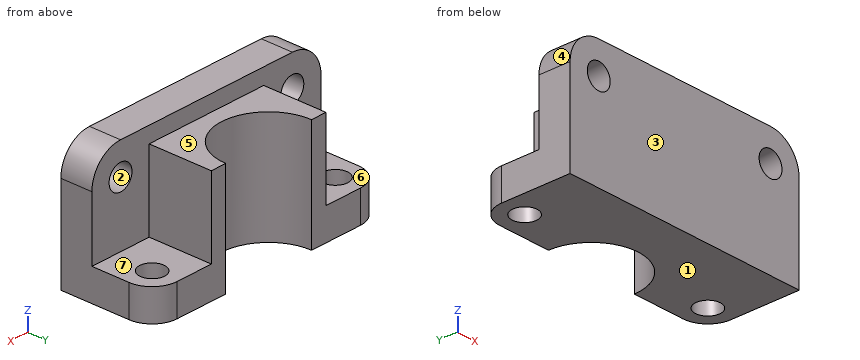
from build123d import *

# Parameters (mm, degrees)
BASE_PLATE_SKETCH_W       = 80
BASE_PLATE_SKETCH_H       = 40
BASE_PLATE_80X40X10_DEPTH = 10
BASE_CORNER_FILLETS_R10_R = 10
SADDLE_BLOCK_DEPTH        = 35
LUG_PROFILE_SKETCH_W      = 20
LUG_PROFILE_SKETCH_H      = 20
UPRIGHT_LUGS_DEPTH        = 10
LUG_TOP_FILLETS_R8_R      = 8
LUG_HOLE_SKETCH_R         = 4
LUG_HOLES_8_DEPTH         = 62
BASE_HOLE_SKETCH_R        = 4
BASE_HOLES_8_DEPTH        = 62


with BuildPart() as part:
    # Base Plate Sketch → Base Plate 80x40x10 (new body)
    with BuildSketch(Plane(origin=(0, 0, 0), x_dir=(1, 0, 0), z_dir=(0, 1, 0))):
        Rectangle(BASE_PLATE_SKETCH_W, BASE_PLATE_SKETCH_H)
    extrude(amount=BASE_PLATE_80X40X10_DEPTH)

    # Base Corner Fillets R10
    base_corner_fillets_r10_edges = [part.edges().sort_by_distance(p)[0] for p in [
        (40, 5, 20),
        (-40, 5, 20),
    ]]
    fillet(base_corner_fillets_r10_edges, radius=BASE_CORNER_FILLETS_R10_R)

    # Saddle Block Sketch → Saddle Block (add)
    with BuildSketch(Plane(origin=(0, 0, -20), x_dir=(-1, 0, 0), z_dir=(0, 0, -1))):
        with BuildLine():
            Line((-20, 10), (20, 10))
            Line((20, 10), (20, 30))
            Line((20, 30), (15, 30))
            ThreePointArc((15, 30), (0, 15), (-15, 30))
            Line((-15, 30), (-20, 30))
            Line((-20, 30), (-20, 10))
        make_face()
    extrude(amount=-SADDLE_BLOCK_DEPTH)

    # Lug Profile Sketch → Upright Lugs (add)
    with BuildSketch(Plane(origin=(0, 0, -20), x_dir=(-1, 0, 0), z_dir=(0, 0, -1))):
        with Locations((-30, 20)):
            Rectangle(LUG_PROFILE_SKETCH_W, LUG_PROFILE_SKETCH_H)
        with Locations((30, 20)):
            Rectangle(LUG_PROFILE_SKETCH_W, LUG_PROFILE_SKETCH_H)
    extrude(amount=-UPRIGHT_LUGS_DEPTH)

    # Lug Top Fillets R8
    lug_top_fillets_r8_edges = [part.edges().sort_by_distance(p)[0] for p in [
        (40, 30, -15),
        (-40, 30, -15),
    ]]
    fillet(lug_top_fillets_r8_edges, radius=LUG_TOP_FILLETS_R8_R)

    # Lug Hole Sketch → Lug Holes Ø8 (cut)
    with BuildSketch(Plane(origin=(0, 0, -20), x_dir=(-1, 0, 0), z_dir=(0, 0, -1))):
        with Locations((32, 22)):
            Circle(LUG_HOLE_SKETCH_R)
        with Locations((-32, 22)):
            Circle(LUG_HOLE_SKETCH_R)
    extrude(amount=-LUG_HOLES_8_DEPTH, mode=Mode.SUBTRACT)

    # Base Hole Sketch → Base Holes Ø8 (cut)
    with BuildSketch(Plane(origin=(0, 10, 0), x_dir=(1, 0, 0), z_dir=(0, 1, 0))):
        with Locations(Location((-30, -10, 0), (0, 0, 270))):
            Circle(BASE_HOLE_SKETCH_R)
        with Locations(Location((30, -10, 0), (0, 0, 270))):
            Circle(BASE_HOLE_SKETCH_R)
    extrude(amount=-BASE_HOLES_8_DEPTH, mode=Mode.SUBTRACT)


solid = part.part
CAD build for the part. Positions are in the model's coordinates, mm. Face numbers are marked on the shaded views. A direction names the side the tool comes from. Coordinates: 2 decimals unless noted, no trailing zeros. Loops run counter-clockwise (first coordinate to the right, second up) from the corner with the lowest first, then second, coordinate; pieces in that order, holes last. Notation, with made-up numbers: (68.25, 15.5) - (104.25, 15.5) arc R21 cw to (104.25, 48.5) - close; hole circle Ø9 at (-33, 60). An arc over 180 degrees is marked (long way). Use one line per item in the form item = value. Start each with the question number.
1) Band-saw the part on D-D (x = 0). Give the cut face in (y, z).
2) Flat gauge pins, fed straight in: pin 1 (9 mm diameter, centred on x = 30, z = 10, fed in from +Y); pin 2 (4 mm diameter, centred on y = 20.5, z = 3, fed in from +X); pin 3 (10 mm diameter, centred on y = 13.5, z = 15.5, fed in from +X). Where does each tip first touch, or does it go through?
3) Band-saw the part on C-C (z = -1.5). Give the cut face in (x, y).
4) Tool access for the marked faces 5, 6 and 7: list every direction of +Z, -Z, +X, -X, +Y, -Y with a clear straight run to the whole face (end or side of a thin tool).
5) Two-plate mould, pull along Z, no slides. Class the marked faces 1, 2, 3 and 4: +Z half, -Z half, draft (parallel to the pull), parting line (faces both ways), or undercut.
6) Drill centre lines: L1, parallel to Y at x = -32, z = -15.5; L2, parallel to Z at x = 35, y = 15; L3, parallel to Z at x = 0, y = 11.75. Where is each one in solid material? Low to high. Write a range as from..to.
7) Band-saw the part on B-B (y = 16.25). Give the cut face in (x, z), and give its area (3 significant figures).
8) Band-saw the part on A-A (z = 12). Give the cut face in (x, y).
Check values:
q1.outline = (0, -20) - (15, -20) - (15, 15) - (10, 15) - (10, 20) - (0, 20) - close
q2.pin_1 = 10
q2.pin_2 = 20
q2.pin_3 = 39.81
q3.outline = (-40, 0) - (40, 0) - (40, 10) - (20, 10) - (20, 30) - (15, 30) arc R15 cw to (-15, 30) - (-20, 30) - (-20, 10) - (-40, 10) - close
q4.face_5 = +Z, +X, -X, +Y
q4.face_6 = +Z, -X, +Y
q4.face_7 = +Z, +X, +Y
q5.face_1 = -Z half
q5.face_2 = undercut
q5.face_3 = draft
q5.face_4 = +Z half
q6.L1 = 0..18, 26..30
q6.L2 = -20..-10
q6.L3 = -20..15
q7.outline = (-40, -20) - (-5.99, -20) - (-5.99, 15) - (-20, 15) - (-20, -10) - (-40, -10) - close; (5.99, -20) - (40, -20) - (40, -10) - (20, -10) - (20, 15) - (5.99, 15) - close
q7.area = 1,380 mm2
q8.outline = (-39.8, 0) - (-33.46, 0) - (-33.46, 10) - (-39.8, 10) - close; (-26.54, 0) - (26.54, 0) - (26.54, 10) - (20, 10) - (20, 30) - (15, 30) arc R15 cw to (-15, 30) - (-20, 30) - (-20, 10) - (-26.54, 10) - close; (33.46, 0) - (39.8, 0) - (39.8, 10) - (33.46, 10) - close
